Geometry check sheet. Reference: the model listing, model coordinates, mm. Face numbers are marked on the shaded views. Round coordinates to 2 decimals unless told otherwise and drop trailing zeros. Write each loop counter-clockwise with the first axis right and the second up, starting at its lowest first coordinate (ties: lowest second). Pieces come first, ordered by that corner, then holes. Notation, with made-up numbers: M 45.5,-16 L 81.5,-16 A32 cw 81.5,13 Z; hole C 73.25,40.5 d2. An arc over 180 degrees is marked long. One line per item, written item: value. Start each with the question number.
1. Section check A-A (y = 0). Record the boundary of the cut face in (x, z).
2. Scan lines: probe 1 along X at (y, z) = (0, -5.5); probe 2 along Z at (x, y) = (4.2, 0); probe 3 along X at (y, z) = (3.8, -3). Record each from-to range of solid material in increasing order. Write a range as [from, to].
3. Release check for a two-part mould opening along Y. For the marked faces 1, 2 and 3 record: pulls with the +Y half, pulls with the -Y half, needs draft (parallel to the pull), parting line crosses it, or undercut.
4. Section check C-C (z = -3). Record the boundary of the cut face in (x, y), and give its area (3 significant figures).
5. Section check D-D (z = -9.5). Record the boundary of the cut face in (x, y), and give its area (3 significant figures).
6. Depth check by flat-ended pin: P1, Ø2, axis at x = 0, z = -3, coming from the +Y side; P2, Ø3, axis at x = 0, y = 0, coming from the +Z side; P3, Ø1.5, axis at x = 2, z = -7, coming from the -Y side; P4, Ø3, axis at y = 3, z = -1.5, coming from the -X side. Enter the tip coordinate at first touch or a pass-through.
from build123d import *

# Parameters (mm, degrees)
SKETCH3_W = 1.25
SKETCH3_H = 5.73
SKETCH5_W = 1.25
SKETCH5_H = 5.73


with BuildPart() as part:
    # Sketch1 → Revolve1 (revolve)
    with BuildSketch(Plane(origin=(0, 0, 0), x_dir=(1, 0, 0), z_dir=(0, 1, 0))):
        Polygon((2.7, 0), (5.53, 0), (5.73, 0.2), (5.73, 11.8), (5.53, 12), (2.7, 12), (2.5, 11.8), (2.5, 0.2), align=None)
    revolve(axis=Axis((0, 0, 0), (0, 0, -1)))

    # Sketch3 → M3 Tapped Hole1 (revolve, cut)
    with BuildSketch(Plane(origin=(0, 0, -3), x_dir=(0, 0, -1), z_dir=(1, 0, 0))):
        with Locations((0.625, 2.865)):
            Rectangle(SKETCH3_W, SKETCH3_H)
    revolve(axis=Axis((0, -6.35, -3), (0, 1, 0)), mode=Mode.SUBTRACT)

    # Sketch5 → M3 Tapped Hole2 (revolve, cut)
    with BuildSketch(Plane(origin=(0, 0, -3), x_dir=(0, 0, 1), z_dir=(0, 1, 0))):
        with Locations((0.625, 2.865)):
            Rectangle(SKETCH5_W, SKETCH5_H)
    revolve(axis=Axis((-6.35, 0, -3), (1, 0, 0)), mode=Mode.SUBTRACT)


solid = part.part
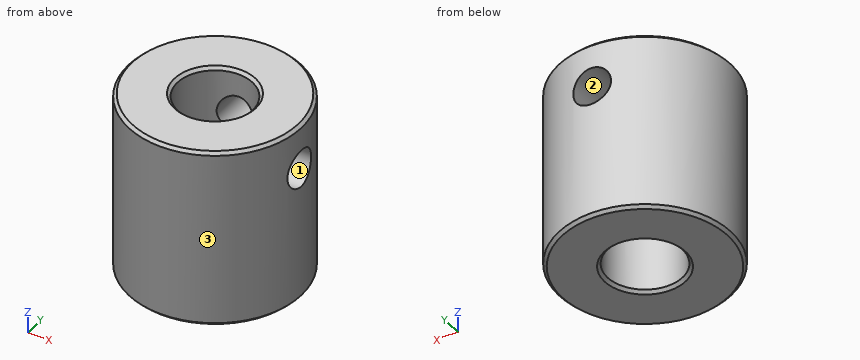
Result sheet:
1. outline: M -5.73,-11.8 L -5.53,-12 L -2.7,-12 L -2.5,-11.8 L -2.5,-0.2 L -2.7,0 L -5.53,0 L -5.73,-0.2 Z; M 2.5,-11.8 L 2.7,-12 L 5.53,-12 L 5.73,-11.8 L 5.73,-4.25 L 2.5,-4.25 Z; M 2.5,-1.75 L 5.73,-1.75 L 5.73,-0.2 L 5.53,0 L 2.7,0 L 2.5,-0.2 Z
2. probe 1: x = [-5.73, -2.5], [2.5, 5.73]
2. probe 2: z = [-12, -4.25], [-1.75, 0]
2. probe 3: x = [-4.29, -1.25], [1.25, 4.29]
3. face 1: undercut
3. face 2: needs draft
3. face 3: parting line crosses it
4. outline: M -1.25,2.17 L -1.25,5.59 A5.73 ccw long 5.59,-1.25 L 2.17,-1.25 A2.5 cw long Z; M 1.25,2.17 A2.5 cw 2.17,1.25 L 5.59,1.25 A5.73 ccw 1.25,5.59 Z
4. area: 67.0 mm2
5. outline: C 0,0 d11.46; hole C 0,0 d5
5. area: 83.5 mm2
6. P1: stops at y = -2.29
6. P2: passes through
6. P3: stops at y = -5.59
6. P4: stops at x = -5.53
